from build123d import *

# Parameters (mm, degrees)
BOSS_EXTRUDE1_DEPTH = 5
FILLET1_R           = 6


with BuildPart() as part:
    # Sketch1 → Boss-Extrude1 (new body)
    with BuildSketch(Plane.XY):
        Polygon((0, 0), (0, 1105.5), (-253.62, 1105.5), (-651, 960.865508307), (-651, 0), align=None)
    extrude(amount=BOSS_EXTRUDE1_DEPTH)

    # Fillet1
    fillet1_edges = [part.edges().sort_by_distance(p)[0] for p in [
        (-651, 960.865508307, 2.5),
        (-253.62, 1105.5, 2.5),
    ]]
    fillet(fillet1_edges, radius=FILLET1_R)


solid = part.part
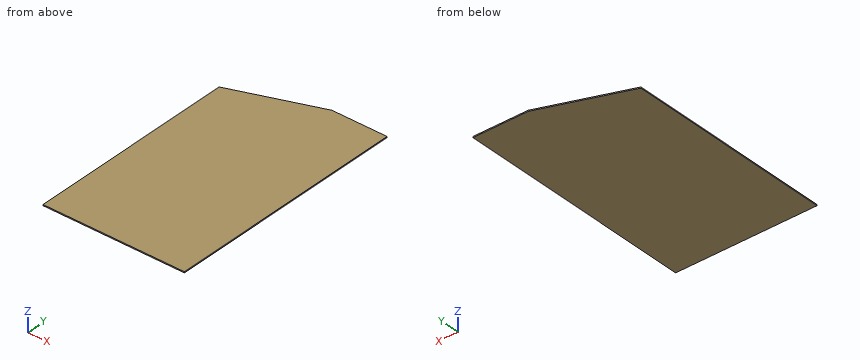
The model under review builds one solid part; all positions refer to its coordinate system, in mm. Give positions to 0.01 mm unless a question says otherwise; leave off trailing zeros. Write each loop counter-clockwise with the first axis right and the second up, starting at its lowest first coordinate (ties: lowest second). Pieces come first, ordered by that corner, then holes.
1. Wall thickness on L1, parallel to Y at x = -589.5, z = 2.6; L2, parallel to Y at x = -281.5, z = 4.45: over which ranges is each line inside the solid? List them lowest first.
2. Add section C-C, the plane x = -607.5. Write out the cut boundary in (y, z).
3. Add section B-B, the plane x = -372. Write out the cut boundary in (y, z).
4. Add section A-A, the plane z = 2.6. Write out the cut boundary in (x, y), plus the area to 3 significant figures.
Worked answers:
1. L1: y = 0 to 983.25
1. L2: y = 0 to 1095.35
2. outline: (0, 0) - (976.7, 0) - (976.7, 5) - (0, 5) - close
3. outline: (0, 0) - (1062.41, 0) - (1062.41, 5) - (0, 5) - close
4. outline: (-651, 0) - (0, 0) - (0, 1105.5) - (-252.56, 1105.5) arc R6 ccw to (-254.61, 1105.14) - (-647.05, 962.3) arc R6 ccw to (-651, 956.66) - close
4. area: 691,000 mm2
